The listing builds one solid part. Answer for the finished solid, in the listing's coordinates (mm). A direction names the side the tool comes from. Coordinates: 2 decimals unless noted, no trailing zeros. Order: outer loops, then holes, each group sorted by start corner. A loop starts at its lowest first (then second) coordinate and runs counter-clockwise, first axis right, second up. Notation, with made-up numbers: (-3, -35.75) -> (2, -35.75) arc R15 ccw to (2, -30.75) -> close; hole circle Ø5 at (-2, 6.25). An arc over 180 degrees is marked (long way). Return JSON: item names as keys, results as strings.
from build123d import *

# Parameters (mm, degrees)
SKETCH_1_W          = 172
SKETCH_1_H          = 42.5
EXTRUDE_2_DEPTH     = 120
CUT_EXTRUDE_1_DEPTH = 35
SKETCH_5_R          = 8
SKETCH_5_R_2        = 4
CUT_EXTRUDE_2_DEPTH = 211.797444244
CUT_EXTRUDE_4_DEPTH = 154.630237909


with BuildPart() as part:
    # 草图1 → 凸台-拉伸2 (new body)
    with BuildSketch(Plane.XY):
        Rectangle(SKETCH_1_W, SKETCH_1_H)
    extrude(amount=EXTRUDE_2_DEPTH)

    # 草图2 → 切除-拉伸1 (cut)
    with BuildSketch(Plane(origin=(0, 21.25, 0), x_dir=(1, 0, 0), z_dir=(0, 1, 0))):
        Polygon((-80, -5), (-80, -3), (80, -3), (80, -5), (80, -117), (-80, -117), align=None)
    extrude(amount=-CUT_EXTRUDE_1_DEPTH, mode=Mode.SUBTRACT)

    # 草图5 → 切除-拉伸2 (cut, through all)
    with BuildSketch(Plane.ZY.offset(86)):
        with Locations((20, 8.75)):
            Circle(SKETCH_5_R)
        with Locations((60, 8.75)):
            Circle(SKETCH_5_R_2)
    extrude(amount=-CUT_EXTRUDE_2_DEPTH, mode=Mode.SUBTRACT)

    # 草图6 → 切除-拉伸4 (cut, through all)
    with BuildSketch(Plane.XZ.offset(21.25)):
        with BuildLine():
            Line((-3.517636002, 50.460607986), (-3.517636002, 46.460607986))
            Line((-3.517636002, 46.460607986), (2.482363998, 46.460607986))
            Line((2.482363998, 46.460607986), (2.482363998, 50.460607986))
            ThreePointArc((2.482363998, 50.460607986), (-0.517636002, 70), (-3.517636002, 50.460607986))
        make_face()
    extrude(amount=-CUT_EXTRUDE_4_DEPTH, mode=Mode.SUBTRACT)


solid = part.part
1. Determine the mould class of faces 4 (the face through (-86, 0, 59)), 5 (the face through (-3.518, -18, 48)), 6 (the face through (-1, 0, 120)) for opening direction X: pulls with the +X half, pulls with the -X half, needs draft (parallel to the pull), parting line crosses it, or undercut.
Answer block:
{"face 4": "pulls with the -X half", "face 5": "undercut", "face 6": "needs draft"}
2. The part is cut by section D-D on z = 20. Give the vertices of the cut face in (x, y).
Answer block:
{"outline": "(-86, -21.25) -> (86, -21.25) -> (86, 0.75) -> (80, 0.75) -> (80, -13.75) -> (-80, -13.75) -> (-80, 0.75) -> (-86, 0.75) -> close; (-86, 16.75) -> (-80, 16.75) -> (-80, 21.25) -> (-86, 21.25) -> close; (80, 16.75) -> (86, 16.75) -> (86, 21.25) -> (80, 21.25) -> close"}
3. Consider line 1 (Z direction, x = -54, y = -5); line 2 (X direction, y = -3, z = 20); line 3 (X direction, y = -16, z = 49.5). Determine where each line is inside the solid, lowest interval first. Write a range as from..to.
Answer block:
{"line 1": "z = 0..3, 117..120", "line 2": "x = -86..-80, 80..86", "line 3": "x = -86..-3.52, 2.48..86"}
4. For faces 1 (the face through (-1, 0, 0)), 2 (the face through (2.482, -18, 48)), 3 (the face through (80, 4, 61)), determine the directions among +Z, -Z, +X, -X, +Y, -Y from which every point of the face is accessible in a straight line to the end or side of a thin tool.
Answer block:
{"face 1": "-Z, +X, -X, +Y, -Y", "face 2": "+Y, -Y", "face 3": "+Y"}
5. The part is cut by section B-B on y = 8.75. Give the vertices of the cut face in (x, z).
Answer block:
{"outline": "(-86, 0) -> (86, 0) -> (86, 12) -> (80, 12) -> (80, 3) -> (-80, 3) -> (-80, 12) -> (-86, 12) -> close; (-86, 28) -> (-80, 28) -> (-80, 56) -> (-86, 56) -> close; (-86, 64) -> (-80, 64) -> (-80, 117) -> (80, 117) -> (80, 64) -> (86, 64) -> (86, 120) -> (-86, 120) -> close; (80, 28) -> (86, 28) -> (86, 56) -> (80, 56) -> close"}
6. The part is cut by section A-A on z = 60. Give the vertices of the cut face in (x, y).
Answer block:
{"outline": "(-86, -21.25) -> (-10.52, -21.25) -> (-10.52, -13.75) -> (-80, -13.75) -> (-80, 4.75) -> (-86, 4.75) -> close; (-86, 12.75) -> (-80, 12.75) -> (-80, 21.25) -> (-86, 21.25) -> close; (9.48, -21.25) -> (86, -21.25) -> (86, 4.75) -> (80, 4.75) -> (80, -13.75) -> (9.48, -13.75) -> close; (80, 12.75) -> (86, 12.75) -> (86, 21.25) -> (80, 21.25) -> close"}
7. This flat-tipped pin is pushed along its axis until it touches: pin 1 Ø3 at (x, z) = (-67.5, 27.5) entering from +Y. Where does it stop, or does it pass through?
Answer block:
{"pin 1": "stops at y = -13.75"}
8. The part is cut by section C-C on y = 18.5. Give the vertices of the cut face in (x, z), and give its area (3 significant figures).
Answer block:
{"outline": "(-86, 0) -> (86, 0) -> (86, 120) -> (-86, 120) -> close; hole (-80, 3) -> (80, 3) -> (80, 117) -> (-80, 117) -> close", "area": "2,400 mm2"}
